The figure shows three views and two pictorial views of one solid part (mm, origin at its lowest corner). Answer the questions. A direction names the side the tool comes from. Give positions to 0.01 mm unless a question says otherwise; leave off trailing zeros. Order: outer loops, then holes, each group sorted by start corner. A loop starts at its lowest first (then second) coordinate and runs counter-clockwise, first axis right, second up. Notation, with made-up numbers: (81.25, 3) - (133.25, 3) arc R26 ccw to (133.25, 37) - close; hole circle Ø11 at (-38.75, 42). An arc over 180 degrees is marked (long way). Return JSON: item names as keys, results as strings. Group by question number.
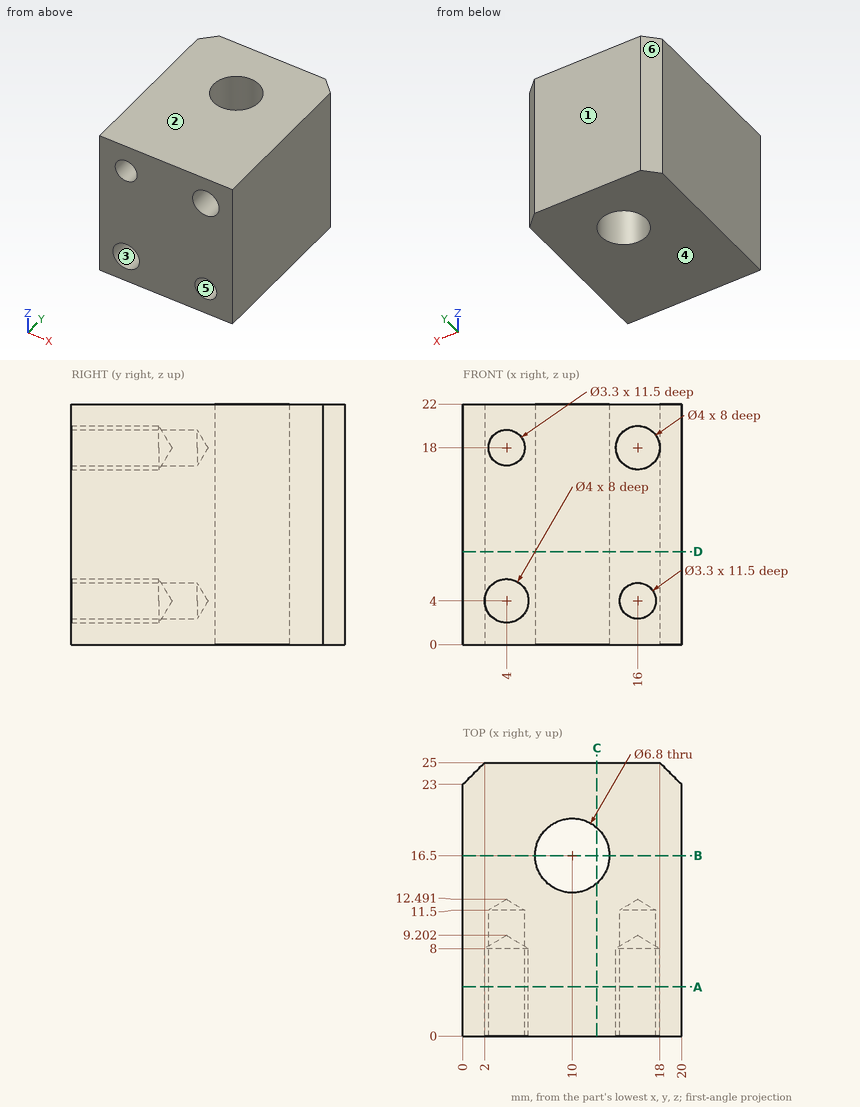
1. The part is cut by section B-B (y = 16.5). Give the vertices of the cut face in (x, z), and give its area (3 significant figures).
2. The part is cut by section D-D (z = 8.5). Give the vertices of the cut face in (x, y).
3. A tool of negligible diameter and unlimited length cuts with its end or side. For the marked faces 5 and 6, from which of +Z, -Z, +X, -X, +Y, -Y can it reach the whole face along a straight path? Write none if from no direction.
4. The part is cut by section A-A (y = 4.5). Give the vertices of the cut face in (x, z).
5. Consider probe 1 along Z at (x, y) = (4, 5); probe 2 along Z at (x, y) = (16, 3.25); probe 3 along X at (y, z) = (5.75, 18). Determine where each line is inside the solid, lowest interval first. Write a range as from..to.
6. The part is cut by section C-C (x = 12.25). Give the vertices of the cut face in (y, z).
7. Determine the mould class of the marked faces 1, 2, 3 and 4 for opening direction Z: released by +Z, released by -Z, zero draft, split by the parting line, or undercut.
8. This flat-tipped pin is pushed along its axis until it touches: pin 1 (3 mm diameter, centred on x = 16, z = 18, fed in from -Y). Where does it stop, or does it pass through?
Answers:
{
 "1": {"outline": "(0, 0) - (6.6, 0) - (6.6, 22) - (0, 22) - close; (13.4, 0) - (20, 0) - (20, 22) - (13.4, 22) - close", "area": "290 mm^2"},
 "2": {"outline": "(0, 0) - (20, 0) - (20, 23) - (18, 25) - (2, 25) - (0, 23) - close; hole circle Ø6.8 at (10, 16.5)"},
 "3": {"face 5": "-Y", "face 6": "+Z, -Z, -X, +Y"},
 "4": {"outline": "(0, 0) - (20, 0) - (20, 22) - (0, 22) - close; hole circle Ø4 at (4, 4); hole circle Ø3.3 at (4, 18); hole circle Ø4 at (16, 18); hole circle Ø3.3 at (16, 4)"},
 "5": {"probe 1": "z = 0..2, 6..16.35, 19.65..22", "probe 2": "z = 0..2.35, 5.65..16, 20..22", "probe 3": "x = 0..2.35, 5.65..14, 18..20"},
 "6": {"outline": "(0, 0) - (13.95, 0) - (13.95, 22) - (0, 22) - close; (19.05, 0) - (25, 0) - (25, 22) - (19.05, 22) - close"},
 "7": {"face 1": "zero draft", "face 2": "released by +Z", "face 3": "undercut", "face 4": "released by -Z"},
 "8": {"pin 1": "stops at y = 8.3"}
}
